```python
from build123d import *

# Parameters (mm, degrees)
CHAMFER_1_SIZE           = 1
SKETCH_4_W               = 10
SKETCH_4_H               = 4.029490121
CUT_EXTRUDE_1_DEPTH      = 69.000919111
CUT_EXTRUDE_3_DEPTH      = 23
CUT_EXTRUDE_3_DEPTH_BACK = 2
SKETCH_6_OUTSIDE_W       = 118.508
SKETCH_6_OUTSIDE_H       = 118.508
SKETCH_6_OUTSIDE_R       = 31.5
SKETCH_9_R               = 32.5
SKETCH_9_R_2             = 31.5
EXTRUDE_1_DEPTH          = 23


with BuildPart() as part:
    # 草图1 → 旋转1 (revolve)
    with BuildSketch(Plane.XY, mode=Mode.PRIVATE) as revolve_1_sk:
        Polygon((0, 17.5), (0, 45.25), (18, 45.25), (18, 31.5), (23, 31.5), (23, 17.5), align=None)
    revolve(revolve_1_sk.sketch.rotate(Axis((0, 0, 0), (1, 0, 0)), 90), axis=Axis((0, 0, 0), (1, 0, 0)))

    # 草图2 → 切除-旋转1 (revolve, cut)
    with BuildSketch(Plane.XY, mode=Mode.PRIVATE) as cut_revolve_1_sk:
        Polygon((11.840143071, 33.8), (15.340759374, 45.25), (2.659240626, 45.25), (6.159856929, 33.8), align=None)
    revolve(cut_revolve_1_sk.sketch.rotate(Axis((0, 0, 0), (1, 0, 0)), 90), axis=Axis((0, 0, 0), (1, 0, 0)), mode=Mode.SUBTRACT)

    # 倒角1
    chamfer_1_edges = [part.edges().sort_by_distance(p)[0] for p in [
        (0, 0, -17.5),
        (23, 0, -17.5),
    ]]
    chamfer(chamfer_1_edges, length=CHAMFER_1_SIZE)

    # 草图4 → 切除-拉伸1 (cut, through all)
    with BuildSketch(Plane.ZY):
        with Locations((0, 18.785254892)):
            Rectangle(SKETCH_4_W, SKETCH_4_H)
    extrude(amount=-CUT_EXTRUDE_1_DEPTH, mode=Mode.SUBTRACT)

    # 草图6 outside → 切除-拉伸3 (cut, two sides: drawn at the far end of the back side and taken through both)
    with BuildSketch(Plane(origin=(0, 0, 0), x_dir=(0, 0, -1), z_dir=(1, 0, 0)).offset(-CUT_EXTRUDE_3_DEPTH_BACK)):
        Rectangle(SKETCH_6_OUTSIDE_W, SKETCH_6_OUTSIDE_H)
        with Locations(Location((0, 0, 0), (0, 0, 180))):
            Circle(SKETCH_6_OUTSIDE_R, mode=Mode.SUBTRACT)
    extrude(amount=CUT_EXTRUDE_3_DEPTH + CUT_EXTRUDE_3_DEPTH_BACK, mode=Mode.SUBTRACT)

    # 草图9 → 凸台-拉伸1 (add)
    with BuildSketch(Plane(origin=(0, 0, 0), x_dir=(0, 0, -1), z_dir=(1, 0, 0))):
        Circle(SKETCH_9_R)
        Circle(SKETCH_9_R_2, mode=Mode.SUBTRACT)
    extrude(amount=EXTRUDE_1_DEPTH)


solid = part.part
```
The listing builds one solid part. Answer for the finished solid, in the listing's coordinates (mm). A direction names the side the tool comes from. Coordinates: 2 decimals unless noted, no trailing zeros. Loops run counter-clockwise (first coordinate to the right, second up) from the corner with the lowest first, then second, coordinate; pieces in that order, holes last. Notation, with made-up numbers: (-13, 48.5) -> (8, 48.5) arc R33 ccw to (8, 85.5) -> close; hole circle Ø1 at (-21, 20). An arc over 180 degrees is marked (long way). Return JSON: item names as keys, results as strings. Group by question number.
(1) A cutting plane is placed at A-A on y = 0. Write down the section's boundary in (x, z), and give its area (3 significant figures).
(2) A cutting plane is placed at B-B on x = 9.5. Write down the section's boundary in (y, z).
(3) A cutting plane is placed at C-C on z = 0. Write down the section's boundary in (x, y).
(4) A cutting plane is placed at D-D on y = 25. Write down the section's boundary in (x, z), and give its area (3 significant figures).
(5) Which of the six approach directions +Z, -Z, +X, -X, +Y, -Y give full straight-line access (tool end or side, diameter ignored) to faces 5 (the flat face through (11, 20.8, 0)), 6 (the flat face through (23, -14, -14))?
(6) Determine the mould class of faces 1 (the flat face through (11, 19, 5)), 2 (the flat face through (0, -14, -14)), 3 (the conical face through (22.174, -17.659, 0.709)), 4 (the cylindrical face through (11.34, 9.76, -31)) for opening direction Z: released by +Z, released by -Z, zero draft, split by the parting line, or undercut.
(7) Find the intervals of material crossed by probe 1 along Y at (x, z) = (11.75, 0); probe 2 along Z at (x, y) = (3, -0.5); probe 3 along Y at (x, z) = (21.25, 12), in increasing order. Write a range as from..to.
(8) Given pin 1 Ø3 at (x, y) = (8.5, 19.5) entering from +Z; pin 2 Ø10 at (x, z) = (13.5, 14.5) entering from -Y; pin 3 Ø3 at (x, z) = (18, -17.5) entering from -Y, each flat-ended and moving along its own axis, determine where each tip first touches the part or whether it passes through.
The answers:
{
 "1": {"outline": "(0, -32.5) -> (23, -32.5) -> (23, -18.5) -> (22, -17.5) -> (1, -17.5) -> (0, -18.5) -> close; (0, 18.5) -> (1, 17.5) -> (22, 17.5) -> (23, 18.5) -> (23, 32.5) -> (0, 32.5) -> close", "area": "688 mm^2"},
 "2": {"outline": "circle Ø65 at (0, 0); hole (16.77, -5) -> (20.8, -5) -> (20.8, 5) -> (16.77, 5) arc R17.5 ccw (long way) to start"},
 "3": {"outline": "(0, -32.5) -> (23, -32.5) -> (23, -18.5) -> (22, -17.5) -> (1, -17.5) -> (0, -18.5) -> close; (0, 20.8) -> (23, 20.8) -> (23, 32.5) -> (0, 32.5) -> close"},
 "4": {"outline": "(0, -20.77) -> (23, -20.77) -> (23, 20.77) -> (0, 20.77) -> close", "area": "955 mm^2"},
 "5": {"face 5": "+X, -X", "face 6": "+Z, -Z, +X, +Y, -Y"},
 "6": {"face 1": "undercut", "face 2": "zero draft", "face 3": "undercut", "face 4": "split by the parting line"},
 "7": {"probe 1": "y = -32.5..-17.5, 20.8..32.5", "probe 2": "z = -32.5..-17.49, 17.49..32.5", "probe 3": "y = -30.2..-12.74, 12.74..30.2"},
 "8": {"pin 1": "stops at z = 27.06", "pin 2": "stops at y = -31.08", "pin 3": "stops at y = -28.29"}
}
